```python
from build123d import *

# Parameters (mm, degrees)
SKETCH_1_W          = 50
SKETCH_1_H          = 70
EXTRUDE_1_DEPTH     = 50
SKETCH_2_R          = 12.5
CUT_EXTRUDE_1_DEPTH = 66.954529791
SKETCH_12_R         = 4
CUT_EXTRUDE_5_DEPTH = 58
CHAMFER_1_SIZE      = 2
CUT_EXTRUDE_START   = -13.5
CUT_EXTRUDE_6_DEPTH = 3


with BuildPart() as part:
    # 草图1 → 凸台-拉伸1 (new body)
    with BuildSketch(Plane.XY):
        Rectangle(SKETCH_1_W, SKETCH_1_H)
    extrude(amount=EXTRUDE_1_DEPTH)

    # 草图2 → 切除-拉伸1 (cut, through all)
    with BuildSketch(Plane.XY.offset(50)):
        Circle(SKETCH_2_R)
    extrude(amount=-CUT_EXTRUDE_1_DEPTH, mode=Mode.SUBTRACT)

    # 草图12 → 切除-拉伸5 (cut)
    with BuildSketch(Plane(origin=(25, 0, 0), x_dir=(0, 0, -1), z_dir=(1, 0, 0))):
        with Locations((-25, 25)):
            Circle(SKETCH_12_R)
    cut_extrude_5 = extrude(amount=-CUT_EXTRUDE_5_DEPTH, mode=Mode.SUBTRACT)

    # 镜向1: 切除-拉伸5 across plane
    add(cut_extrude_5.mirror(Plane.ZX), mode=Mode.SUBTRACT)

    # 倒角1
    chamfer_1_edges = [part.edges().sort_by_distance(p)[0] for p in [
        (-25, 0, 50),
        (0, -35, 50),
        (25, 0, 50),
        (0, -35, 0),
        (-25, 0, 0),
        (0, 35, 0),
        (25, 0, 0),
        (25, -35, 25),
        (-25, -35, 25),
        (-25, 35, 25),
        (25, 35, 25),
        (0, 35, 50),
    ]]
    chamfer(chamfer_1_edges, length=CHAMFER_1_SIZE)

    # 草图13 → 切除-拉伸6 (cut)
    with BuildSketch(Plane(origin=(25, 0, 0), x_dir=(0, 0, -1), z_dir=(1, 0, 0)).offset(CUT_EXTRUDE_START)):
        with BuildLine():
            Line((-50, 5), (-28, 5))
            ThreePointArc((-28, 5), (-23, 0), (-28, -5))
            Line((-28, -5), (-50, -5))
            ThreePointArc((-50, -5), (-55, 0), (-50, 5))
        make_face()
    extrude(amount=CUT_EXTRUDE_6_DEPTH, mode=Mode.SUBTRACT)


solid = part.part
```
Verification items for the finished model (mm, model axes). A direction names the side the tool comes from. Give positions to 0.01 mm unless a question says otherwise; leave off trailing zeros. Order: outer loops, then holes, each group sorted by start corner. A loop starts at its lowest first (then second) coordinate and runs counter-clockwise, first axis right, second up. Notation, with made-up numbers: (83.25, 76.5) - (117.25, 76.5) arc R26 cw to (117.25, 114.5) - close; hole circle Ø5 at (-26.5, -20.5). An arc over 180 degrees is marked (long way). Answer as CSV lines item,"result". Start each with the question number.
Item 1: Section check B-B, the plane x = 0. Record the boundary of the cut face in (y, z).
Item 2: Section check D-D, the plane z = 40. Record the boundary of the cut face in (x, y).
Item 3: Material ranges on L1, parallel to Y at x = -14.5, z = 25; L2, parallel to Y at x = 0, z = 12; L3, parallel to Y at x = -11, z = 26, recorded low to high.
Item 4: Section check C-C, the plane x = -13.5. Record the boundary of the cut face in (y, z).
Item 5: Access from +Z, -Z, +X, -X, +Y, -Y to the whole of each face (thin tool, end or side, straight path). Record for faces 1 (the face through (-23.6, -33.8, 48.6)), 2 (the face through (13, 5, 39)).
Item 6: Gauge pin test, flat end, axial feed: pin 1 (6.5 mm diameter, centred on y = 25, z = 25, fed in from +X). Record the tip position at first contact, or that the pin passes through.
Item 7: Section check A-A, the plane y = -25. Record the boundary of the cut face in (x, z), plus the area to 3 significant figures.
Item 8: Mould release check, pull along Y, two halves, no side actions. Record for faces 3 (the face through (0, -34, 49)), 4 (the face through (-23.6, 33.8, 48.6)), 5 (the face through (13, -5, 39)): released by +Y, released by -Y, zero draft, split by the parting line, or undercut.
Filled in:
1,outline,"(-35, 2) - (-33, 0) - (-12.5, 0) - (-12.5, 50) - (-33, 50) - (-35, 48) - close; (12.5, 0) - (33, 0) - (35, 2) - (35, 48) - (33, 50) - (12.5, 50) - close; hole circle Ø8 at (-25, 25); hole circle Ø8 at (25, 25)"
2,outline,"(-25, -33) - (-23, -35) - (23, -35) - (25, -33) - (25, 33) - (23, 35) - (-23, 35) - (-25, 33) - close; hole (11.5, -5) - (14.5, -5) - (14.5, 5) - (11.5, 5) - (11.5, 4.9) arc R12.5 ccw (long way) to (11.5, -4.9) - close"
3,L1,"-35 to -29, -21 to 21, 29 to 35"
3,L2,"-35 to -12.5, 12.5 to 35"
3,L3,"-35 to -28.87, -21.13 to -5.94, 5.94 to 21.13, 28.87 to 35"
4,outline,"(-35, 2) - (-33, 0) - (33, 0) - (35, 2) - (35, 48) - (33, 50) - (-33, 50) - (-35, 48) - close; hole circle Ø8 at (-25, 25); hole circle Ø8 at (25, 25)"
5,face 1,"+Z, -X, -Y"
5,face 2,"+Z"
6,pin 1,"through"
7,outline,"(-25, 2) - (-23, 0) - (23, 0) - (25, 2) - (25, 21) - (-25, 21) - close; (-25, 29) - (25, 29) - (25, 48) - (23, 50) - (-23, 50) - (-25, 48) - close"
7,area,"2,090 mm^2"
8,face 3,"released by -Y"
8,face 4,"released by +Y"
8,face 5,"undercut"
